Geometry: see drawing. Coordinates: mm, zero at the bounding-box minimum. A direction names the side the tool comes from. Give positions to 0.01 mm unless a question says otherwise; leave off trailing zeros. Write each loop counter-clockwise with the first axis right and the second up, starting at its lowest first coordinate (ties: lowest second). Pieces come first, ordered by that corner, then holes. Notation, with made-up numbers: M 80,15 L 90,15 A20 ccw 90,24 Z; hole C 87.25,64 d7. An arc over 180 degrees is marked long. Answer as a JSON object with one key per item and string values. Group by question number.
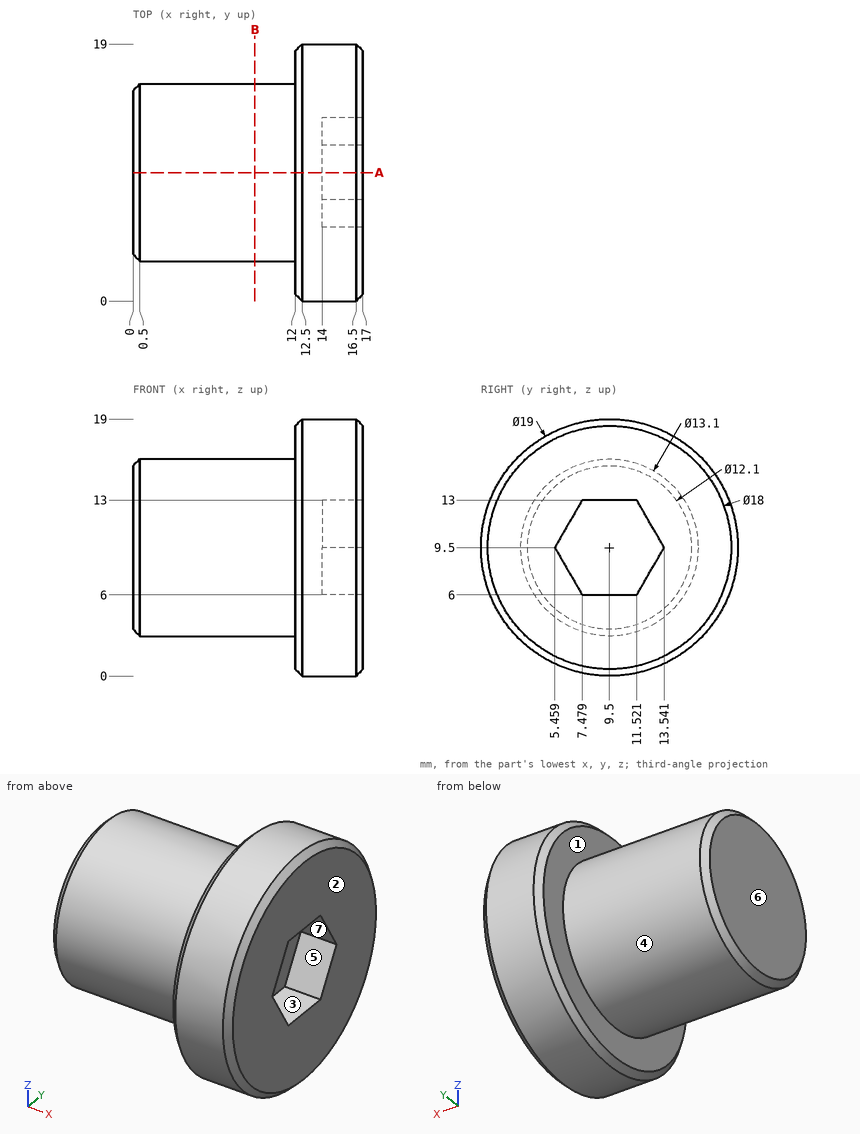
(1) Pull-direction query (Z, two-part tool) for the marked faces 4, 5, 6 and 7; classes: pulls with the +Z half, pulls with the -Z half, needs draft (parallel to the pull), parting line crosses it, or undercut.
(2) Contact query for flat-ended pins moving along their axis: pin 1 Ø0.9 at (x, y) = (15.5, 8.5) entering from -Z; pin 2 Ø3 at (x, y) = (11, 16) entering from +Z; pin 3 Ø2 at (x, y) = (10, 10) entering from -Z. Output: stop coordinate, or through.
(3) Access query for the marked faces 1, 2 and 3. Directions: +Z, -Z, +X, -X, +Y, -Y. A direction counts if a zero-diameter tool reaches every point of the face in a straight line with its end or side. Return the directions, or none.
(4) Section A-A, the plane y = 9.5. Return loops of the section in (x, z).
(5) Ray query, L1, parallel to X at y = 2.25, z = 7.25; L2, parallel to X at y = 8, z = 12.5; L3, parallel to Y at x = 15.25, z = 12.25 (1 decimal). Return the intervals inside material, ascending. Write a range as [from, to].
(6) Section B-B, the plane x = 9. Return loops of the section in (y, z).
Reported:
{
 "1": {"face 4": "parting line crosses it", "face 5": "undercut", "face 6": "needs draft", "face 7": "undercut"},
 "2": {"pin 1": "stops at z = 0.02", "pin 2": "stops at z = 16.81", "pin 3": "stops at z = 2.95"},
 "3": {"face 1": "-X", "face 2": "+Z, -Z, +X, +Y, -Y", "face 3": "+X"},
 "4": {"outline": "M 0,3.45 L 0.5,2.95 L 12,2.95 L 12,0.5 L 12.5,0 L 16.5,0 L 17,0.5 L 17,6 L 14,6 L 14,13 L 17,13 L 17,18.5 L 16.5,19 L 12.5,19 L 12,18.5 L 12,16.05 L 0.5,16.05 L 0,15.55 Z"},
 "5": {"L1": "x = [12, 17]", "L2": "x = [0, 14]", "L3": "y = [0.4, 7], [12, 18.6]"},
 "6": {"outline": "C 9.5,9.5 d13.1"}
}
